```python
from build123d import *

# Parameters (mm, degrees)
SKETCH1_W           = 35
SKETCH1_H           = 44
SKETCH1_W_2         = 31
SKETCH1_H_2         = 40
BOSS_EXTRUDE1_DEPTH = 488.48935286


with BuildPart() as part:
    # Sketch1 → Boss-Extrude1 (new body)
    with BuildSketch(Plane.XY):
        Rectangle(SKETCH1_W, SKETCH1_H)
        Rectangle(SKETCH1_W_2, SKETCH1_H_2, mode=Mode.SUBTRACT)
    extrude(amount=BOSS_EXTRUDE1_DEPTH)


solid = part.part
```
Part model, mm, in its own coordinate system. A direction names the side the tool comes from. Give positions to 0.01 mm unless a question says otherwise; leave off trailing zeros. Write each loop counter-clockwise with the first axis right and the second up, starting at its lowest first coordinate (ties: lowest second). Pieces come first, ordered by that corner, then holes. Notation, with made-up numbers: (54.5, 65) -> (107.5, 65) arc R35 cw to (107.5, 100) -> close; hole circle Ø4 at (68, -28.75). An arc over 180 degrees is marked (long way). Put each result on its own line as item: value. Start each with the question number.
Item 1: Pull direction Y, two halves, no side cores. Call faces 3 (the face through (0, -20, 241)), 4 (the face through (0, -22, 241)), 5 (the face through (-16, 0, 0)): pulls with the +Y half, pulls with the -Y half, needs draft (parallel to the pull), parting line crosses it, or undercut.
Item 2: Cut at A-A (x = -10). List the corners of the cut face in (y, z).
Item 3: Wall check: L1, parallel to X at y = 1, z = 293; L2, parallel to Y at x = 5.5, z = 281. Give the ranges that are in metal, low to high. Write a range as [from, to].
Item 4: Cut at B-B (y = -0.5). List the corners of the cut face in (x, z).
Item 5: Which spindle directions (+Z, -Z, +X, -X, +Y, -Y) get a long thin tool onto all of the face, cutting with end or side? Do faces 1 (the face through (15.5, 0, 241)), 2 (the face through (-17.5, 0, 241)). Say none if no direction does.
Item 6: Cut at C-C (z = 387.5). List the corners of the cut face in (x, y), then the cut area to 3 significant figures.
Answer list:
1. face 3: undercut
1. face 4: pulls with the -Y half
1. face 5: needs draft
2. outline: (-22, 0) -> (-20, 0) -> (-20, 488.49) -> (-22, 488.49) -> close; (20, 0) -> (22, 0) -> (22, 488.49) -> (20, 488.49) -> close
3. L1: x = [-17.5, -15.5], [15.5, 17.5]
3. L2: y = [-22, -20], [20, 22]
4. outline: (-17.5, 0) -> (-15.5, 0) -> (-15.5, 488.49) -> (-17.5, 488.49) -> close; (15.5, 0) -> (17.5, 0) -> (17.5, 488.49) -> (15.5, 488.49) -> close
5. face 1: +Z, -Z
5. face 2: +Z, -Z, -X, +Y, -Y
6. outline: (-17.5, -22) -> (17.5, -22) -> (17.5, 22) -> (-17.5, 22) -> close; hole (-15.5, -20) -> (15.5, -20) -> (15.5, 20) -> (-15.5, 20) -> close
6. area: 300 mm2
